Could you check a few things on this drawing? It's one solid part, dimensions in mm from its lowest x, y, z. A direction names the side the tool comes from. Round coordinates to 2 decimals unless told otherwise and drop trailing zeros. Write each loop counter-clockwise with the first axis right and the second up, starting at its lowest first coordinate (ties: lowest second). Pieces come first, ordered by that corner, then holes. Notation, with made-up numbers: (38, -8.75) -> (72, -8.75) arc R16 cw to (72, 18.25) -> close; hole circle Ø5 at (84, 77.5). An arc over 180 degrees is marked (long way). Return JSON: item names as keys, results as strings.
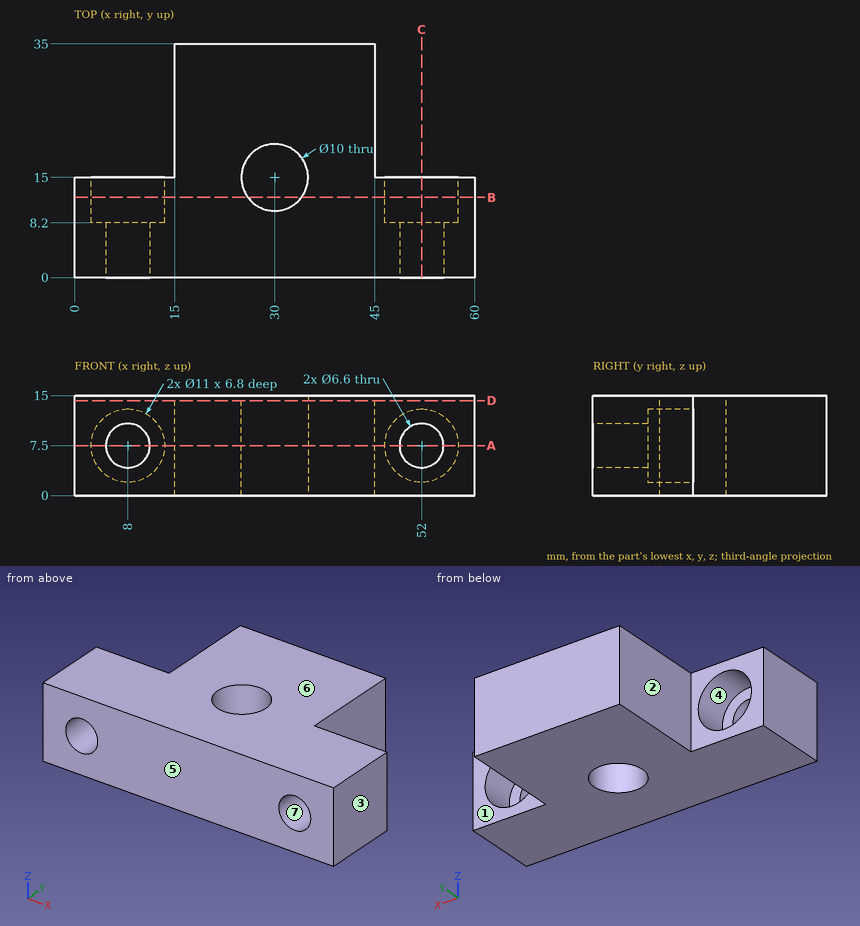
1) I want a section at B-B, the plane y = 12. Please give me the cut outline in (x, z), and give its area (3 significant figures).
Return value:
{"outline": "(0, 0) -> (26, 0) -> (26, 15) -> (0, 15) -> close; (34, 0) -> (60, 0) -> (60, 15) -> (34, 15) -> close; hole circle Ø11 at (8, 7.5); hole circle Ø11 at (52, 7.5)", "area": "590 mm²"}
2) Will these pins go through, and if not, where does the flat tip stop? pin 1 Ø9 at (x, z) = (7, 8) entering from +Y; pin 2 Ø4.5 at (y, z) = (27, 9.5) entering from -X.
Return value:
{"pin 1": "y = 15", "pin 2": "x = 15"}
3) I want a section at A-A, the plane z = 7.5. Please give me the cut outline in (x, y), and give its area (3 significant figures).
Return value:
{"outline": "(0, 0) -> (4.7, 0) -> (4.7, 8.2) -> (2.5, 8.2) -> (2.5, 15) -> (0, 15) -> close; (11.3, 0) -> (48.7, 0) -> (48.7, 8.2) -> (46.5, 8.2) -> (46.5, 15) -> (45, 15) -> (45, 35) -> (15, 35) -> (15, 15) -> (13.5, 15) -> (13.5, 8.2) -> (11.3, 8.2) -> close; (55.3, 0) -> (60, 0) -> (60, 15) -> (57.5, 15) -> (57.5, 8.2) -> (55.3, 8.2) -> close; hole circle Ø10 at (30, 15)", "area": "1,160 mm²"}
4) Thinking about a two-plate mould opening in Z: for the marked faces 5, 6 and 7, which applies, pulls with the +Z half, pulls with the -Z half, needs draft (parallel to the pull), parting line crosses it, or undercut?
Return value:
{"face 5": "needs draft", "face 6": "pulls with the +Z half", "face 7": "undercut"}
5) I want a section at D-D, the plane z = 14.25. Please give me the cut outline in (x, y), and give its area (3 significant figures).
Return value:
{"outline": "(0, 0) -> (60, 0) -> (60, 15) -> (45, 15) -> (45, 35) -> (15, 35) -> (15, 15) -> (0, 15) -> close; hole circle Ø10 at (30, 15)", "area": "1,420 mm²"}
6) For the marked faces 1, 2, 3 and 4, which set-ups out of +Z, -Z, +X, -X, +Y, -Y let a thin tool reach every point of the face, with its end or its side?
Return value:
{"face 1": "+Z, -Z, +X, +Y", "face 2": "+Z, -Z, -X, +Y", "face 3": "+Z, -Z, +X, +Y, -Y", "face 4": "+Y"}
7) If I drill on probe 1 along X at (y, z) = (3, 7.5); probe 2 along X at (y, z) = (17.5, 5.25); probe 3 along X at (y, z) = (13, 14.5), over which ranges is the centre line in solid material (lowest first)? Write a range as [from, to].
Return value:
{"probe 1": "[0, 4.7], [11.3, 48.7], [55.3, 60]", "probe 2": "[15, 25.67], [34.33, 45]", "probe 3": "[0, 25.42], [34.58, 60]"}
8) I want a section at C-C, the plane x = 52. Please give me the cut outline in (y, z).
Return value:
{"outline": "(0, 0) -> (15, 0) -> (15, 2) -> (8.2, 2) -> (8.2, 4.2) -> (0, 4.2) -> close; (0, 10.8) -> (8.2, 10.8) -> (8.2, 13) -> (15, 13) -> (15, 15) -> (0, 15) -> close"}
